The listing builds one solid part. Answer for the finished solid, in the listing's coordinates (mm). A direction names the side the tool comes from. Coordinates: 2 decimals unless noted, no trailing zeros. Order: outer loops, then holes, each group sorted by start corner. A loop starts at its lowest first (then second) coordinate and runs counter-clockwise, first axis right, second up. Notation, with made-up numbers: (16.25, 30.25) -> (74.25, 30.25) arc R28 cw to (74.25, 54.25) -> close; hole circle Ø9 at (-4.75, -35.75). An arc over 180 degrees is marked (long way). Return JSON: item names as keys, results as strings.
```python
from build123d import *

# Parameters (mm, degrees)
EXTRUDE_1_DEPTH = 5


with BuildPart() as part:
    # 草图1 → 凸台-拉伸1 (new body)
    with BuildSketch(Plane.XY):
        Polygon((0, 0), (0, 130), (40, 130), (40, 40), (100, 40), (100, 120), (180, 120), (180, 0), align=None)
    extrude(amount=EXTRUDE_1_DEPTH)


solid = part.part
```
Item 1: The part is cut by section A-A on y = 114. Determine the outline of the cut face in (x, z).
Answer list:
{"outline": "(0, 0) -> (40, 0) -> (40, 5) -> (0, 5) -> close; (100, 0) -> (180, 0) -> (180, 5) -> (100, 5) -> close"}
Item 2: Which of the six approach directions +Z, -Z, +X, -X, +Y, -Y give full straight-line access (tool end or side, diameter ignored) to faces 4 (the flat face through (139, 120, 2)), 5 (the flat face through (111, 51, 0)), 6 (the flat face through (100, 79, 2))?
Answer list:
{"face 4": "+Z, -Z, +X, +Y", "face 5": "-Z, +X, -X, +Y, -Y", "face 6": "+Z, -Z, +Y"}
Item 3: The part is cut by section D-D on x = 43. Determine the outline of the cut face in (y, z).
Answer list:
{"outline": "(0, 0) -> (40, 0) -> (40, 5) -> (0, 5) -> close"}
Item 4: Flat-ended cylindrical pins translate along their axes: pin 1 (1 mm diameter, centred on x = 144.5, y = 74, fed in from -Z); pin 2 (3 mm diameter, centred on x = 126, z = 4, fed in from +Y); pin 3 (2.5 mm diameter, centred on x = 82.5, z = 1.5, fed in from +Y). Find the tip coordinate at first contact, or state that the pin passes through.
Answer list:
{"pin 1": "z = 0", "pin 2": "y = 120", "pin 3": "y = 40"}
Item 5: The part is cut by section B-B on z = 2. Determine the outline of the cut face in (x, y).
Answer list:
{"outline": "(0, 0) -> (180, 0) -> (180, 120) -> (100, 120) -> (100, 40) -> (40, 40) -> (40, 130) -> (0, 130) -> close"}
Item 6: The part is cut by section C-C on x = 149.5. Determine the outline of the cut face in (y, z), plus the area to 3 significant figures.
Answer list:
{"outline": "(0, 0) -> (120, 0) -> (120, 5) -> (0, 5) -> close", "area": "600 mm2"}
Item 7: Determine the mould class of faces 1 (the flat face through (40, 86, 2)), 2 (the flat face through (180, 61, 2)), 3 (the flat face through (111, 51, 5)) for opening direction X: pulls with the +X half, pulls with the -X half, needs draft (parallel to the pull), parting line crosses it, or undercut.
Answer list:
{"face 1": "undercut", "face 2": "pulls with the +X half", "face 3": "needs draft"}
Item 8: Find the intervals of material crossed by probe 1 along X at (y, z) = (43.5, 1.4); probe 2 along Y at (x, z) = (166, 4.05); probe 3 along Y at (x, z) = (49.5, 1.25), in increasing order.
Answer list:
{"probe 1": "0 to 40, 100 to 180", "probe 2": "0 to 120", "probe 3": "0 to 40"}
